```python
from build123d import *

# Parameters (mm, degrees)
FEATURE_19_WELDMEMBERFEAT_4_MORE_IN_5_DEPTH = 1340
CUT_EXTRUDE1_DEPTH                          = 1343.283502096
CUT_EXTRUDE1_DEPTH_BACK                     = 1343.283502096


with BuildPart() as part:
    # Sketch1 → feature 19 (WeldMemberFeat) (+4 more in 5 files) Cold-formed Hollow Structural Square Steel(gb t6728-2002) 70×70×5(1) (new body)
    with BuildSketch(Plane(origin=(0, 0, 0), x_dir=(-1, 0, 0), z_dir=(0, 1, 0))):
        with BuildLine():
            Line((-25, -35), (25, -35))
            ThreePointArc((25, -35), (32.071067812, -32.071067812), (35, -25))
            Line((35, -25), (35, 25))
            ThreePointArc((35, 25), (32.071067812, 32.071067812), (25, 35))
            Line((25, 35), (-25, 35))
            ThreePointArc((-25, 35), (-32.071067812, 32.071067812), (-35, 25))
            Line((-35, 25), (-35, -25))
            ThreePointArc((-35, -25), (-32.071067812, -32.071067812), (-25, -35))
        make_face()
        with BuildLine():
            Line((-25, -30), (25, -30))
            ThreePointArc((25, -30), (28.535533906, -28.535533906), (30, -25))
            Line((30, -25), (30, 25))
            ThreePointArc((30, 25), (28.535533906, 28.535533906), (25, 30))
            Line((25, 30), (-25, 30))
            ThreePointArc((-25, 30), (-28.535533906, 28.535533906), (-30, 25))
            Line((-30, 25), (-30, -25))
            ThreePointArc((-30, -25), (-28.535533906, -28.535533906), (-25, -30))
        make_face(mode=Mode.SUBTRACT)
    extrude(amount=FEATURE_19_WELDMEMBERFEAT_4_MORE_IN_5_DEPTH)

    # 0:feat:20/0 feature 20/0 (ProfileFeature) (+11 more in 7 files) Sketch2 → Cut-Extrude1 (cut, two sides: drawn at the far end of the back side and taken through both)
    with BuildSketch(Plane.XY.offset(35).offset(-CUT_EXTRUDE1_DEPTH_BACK)):
        Polygon((35, 1340), (-35, 1252.5), (-35, 1340), align=None)
        Polygon((-35, 56), (35, 0), (-35, 0), align=None)
    extrude(amount=CUT_EXTRUDE1_DEPTH + CUT_EXTRUDE1_DEPTH_BACK, mode=Mode.SUBTRACT)


solid = part.part
```
The listing builds one solid part. Answer for the finished solid, in the listing's coordinates (mm). A direction names the side the tool comes from. Give positions to 0.01 mm unless a question says otherwise; leave off trailing zeros. Order: outer loops, then holes, each group sorted by start corner. A loop starts at its lowest first (then second) coordinate and runs counter-clockwise, first axis right, second up. Notation, with made-up numbers: (41, 36.5) -> (95, 36.5) arc R12 ccw to (95, 51.5) -> close; hole circle Ø5 at (61, 61.5). An arc over 180 degrees is marked (long way). One line per item, written item: value.
1) Flat-ended cylindrical pins translate along their axes: P1, Ø4, axis at y = 395, z = 25.5, coming from the +X side; P2, Ø6, axis at x = 25.5, z = 9.5, coming from the -Y side. Find the tip coordinate at first contact, or state that the pin passes through.
Reported:
P1: stops at x = 35
P2: passes through
2) Find the intervals of material crossed by line 1 (Z direction, x = 11, y = 506); line 2 (X direction, y = 1229, z = 26.5), in increasing order.
Reported:
line 1: z = -35 to -30, 30 to 35
line 2: x = -34.89 to -29.77, 29.77 to 34.89
3) Find section A-A, the plane x = 2. Determine the outline of the cut face in (y, z), plus the area to 3 significant figures.
Reported:
outline: (26.4, -35) -> (1298.75, -35) -> (1298.75, -30) -> (26.4, -30) -> close; (26.4, 30) -> (1298.75, 30) -> (1298.75, 35) -> (26.4, 35) -> close
area: 12,700 mm^2
4) Find section C-C, the plane y = 901.5. Determine the outline of the cut face in (x, z), plus the area to 3 significant figures.
Reported:
outline: (-35, -25) arc R10 ccw to (-25, -35) -> (25, -35) arc R10 ccw to (35, -25) -> (35, 25) arc R10 ccw to (25, 35) -> (-25, 35) arc R10 ccw to (-35, 25) -> close; hole (-30, -25) arc R5 ccw to (-25, -30) -> (25, -30) arc R5 ccw to (30, -25) -> (30, 25) arc R5 ccw to (25, 30) -> (-25, 30) arc R5 ccw to (-30, 25) -> close
area: 1,240 mm^2
5) A tool of negligible diameter and unlimited length cuts with its end or side. For faces 1 (the flat face through (0, 659, -35)), 2 (the flat face through (0, 659, -30)), from which of +Z, -Z, +X, -X, +Y, -Y can it reach the whole face along a straight path? Write none if from no direction.
Reported:
face 1: -Z, +X, -X, +Y, -Y
face 2: +Y, -Y
6) Find section B-B, the plane z = 14. Determine the outline of the cut face in (x, y), plus the area to 3 significant figures.
Reported:
outline: (-35, 56) -> (-30, 52) -> (-30, 1258.75) -> (-35, 1252.5) -> close; (30, 4) -> (35, 0) -> (35, 1340) -> (30, 1333.75) -> close
area: 12,700 mm^2
7) Determine the mould class of faces 3 (the flat face through (30, 660, 0)), 4 (the flat face through (0, 659, 35)), 5 (the flat face through (0, 28, 31)) for opening direction X: pulls with the +X half, pulls with the -X half, needs draft (parallel to the pull), parting line crosses it, or undercut.
Reported:
face 3: undercut
face 4: needs draft
face 5: pulls with the -X half
